Check sheet for the modelled part. Datum: model origin and axes. Units: mm. A direction names the side the tool comes from. Give positions to 0.01 mm unless a question says otherwise; leave off trailing zeros. Write each loop counter-clockwise with the first axis right and the second up, starting at its lowest first coordinate (ties: lowest second). Pieces come first, ordered by that corner, then holes. Notation, with made-up numbers: M 69,65.5 L 120,65.5 A23 cw 120,84.5 Z; hole C 62.5,71.25 d10. An arc over 180 degrees is marked long. Use CSV: the item, a comma, the result in double quotes. Start each with the question number.
1. Scan lines: line 1 (Y direction, x = -1, z = 178.5); line 2 (X direction, y = -0.5, z = 310.5) (3 decimals); line 3 (Z direction, x = 18, y = -8.5). Record each from-to range of solid material in increasing order.
2. Mould release check, pull along Y, two halves, no side actions. Record for faces 1 (the face through (-3.47, -15.62, 183.89)), 2 (the face through (-5.961, -26.846, 27.143)), 3 (the face through (16.3, 0.4, 373)): +Y half, -Y half, draft (parallel to the pull), parting line (faces both ways), or undercut.
3. Depth check by flat-ended pin: P1, Ø12, axis at x = 10, z = 322.5, coming from the +Y side; P2, Ø2, axis at x = -18, y = 11, coming from the +Z side; P3, Ø1.2, axis at x = -20, y = 0, coming from the -Z side. Enter the tip coordinate at first touch or a pass-through.
4. Access from +Z, -Z, +X, -X, +Y, -Y to the whole of each face (thin tool, end or side, straight path). Record for faces 4 (the face through (-0.4, -16.6, 0)), 5 (the face through (23.846, 7.509, 210.76)).
5. Cross-section at A-A, the plane z = 210. Enter the section's corners in (x, y), and give its area (3 significant figures).
from build123d import *

# Parameters (mm, degrees)
SKETCH1_R           = 27.5
SKETCH1_R_2         = 16
BOSS_EXTRUDE1_DEPTH = 53
SKETCH2_R           = 25
SKETCH2_R_2         = 16
BOSS_EXTRUDE2_DEPTH = 70
SKETCH3_R           = 2
CUT_EXTRUDE1_DEPTH  = 15
CHAMFER1_SIZE       = 2
SKETCH4_R           = 25
SKETCH4_R_2         = 16
BOSS_EXTRUDE3_DEPTH = 250
SKETCH5_R           = 2
CUT_EXTRUDE2_DEPTH  = 12


with BuildPart() as part:
    # Sketch1 → Boss-Extrude1 (new body)
    with BuildSketch(Plane.XY):
        Circle(SKETCH1_R)
        Circle(SKETCH1_R_2, mode=Mode.SUBTRACT)
    extrude(amount=BOSS_EXTRUDE1_DEPTH)

    # Sketch2 → Boss-Extrude2 (add)
    with BuildSketch(Plane.XY.offset(53)):
        Circle(SKETCH2_R)
        Circle(SKETCH2_R_2, mode=Mode.SUBTRACT)
    extrude(amount=BOSS_EXTRUDE2_DEPTH)

    # Sketch3 → Cut-Extrude1 (cut)
    with BuildSketch(Plane(origin=(0, 0, 0), x_dir=(-1, 0, 0), z_dir=(0, 0, -1))):
        with Locations((0, 19)):
            Circle(SKETCH3_R)
        with Locations((13.435028843, 13.435028843)):
            Circle(SKETCH3_R)
        with Locations((19, 0)):
            Circle(SKETCH3_R)
        with Locations((13.435028843, -13.435028843)):
            Circle(SKETCH3_R)
        with Locations((0, -19)):
            Circle(SKETCH3_R)
        with Locations((-13.435028843, -13.435028843)):
            Circle(SKETCH3_R)
        with Locations((-19, 0)):
            Circle(SKETCH3_R)
        with Locations((-13.435028843, 13.435028843)):
            Circle(SKETCH3_R)
    extrude(amount=-CUT_EXTRUDE1_DEPTH, mode=Mode.SUBTRACT)

    # Chamfer1
    chamfer1_edges = [part.edges().sort_by_distance(p)[0] for p in [
        (-27.5, 0, 0),
    ]]
    chamfer(chamfer1_edges, length=CHAMFER1_SIZE)

    # Sketch4 → Boss-Extrude3 (add)
    with BuildSketch(Plane.XY.offset(123)):
        Circle(SKETCH4_R)
        Circle(SKETCH4_R_2, mode=Mode.SUBTRACT)
    extrude(amount=BOSS_EXTRUDE3_DEPTH)

    # Sketch5 → Cut-Extrude2 (cut)
    with BuildSketch(Plane.XY.offset(373)):
        with Locations((0, 20.5)):
            Circle(SKETCH5_R)
        with Locations((17.753520778, 10.25)):
            Circle(SKETCH5_R)
        with Locations((17.753520778, -10.25)):
            Circle(SKETCH5_R)
        with Locations((0, -20.5)):
            Circle(SKETCH5_R)
        with Locations((-17.753520778, -10.25)):
            Circle(SKETCH5_R)
        with Locations((-17.753520778, 10.25)):
            Circle(SKETCH5_R)
    extrude(amount=-CUT_EXTRUDE2_DEPTH, mode=Mode.SUBTRACT)


solid = part.part
Worked answers:
1,line 1,"y = -24.98 to -15.97, 15.97 to 24.98"
1,line 2,"x = -24.995 to -15.992, 15.992 to 24.995"
1,line 3,"z = 0 to 361"
2,face 1,"undercut"
2,face 2,"parting line"
2,face 3,"draft"
3,P1,"stops at y = 24.68"
3,P2,"stops at z = 361"
3,P3,"stops at z = 15"
4,face 4,"-Z, +X, -X, +Y, -Y"
4,face 5,"+Z"
5,outline,"C 0,0 d50; hole C 0,0 d32"
5,area,"1,160 mm^2"
